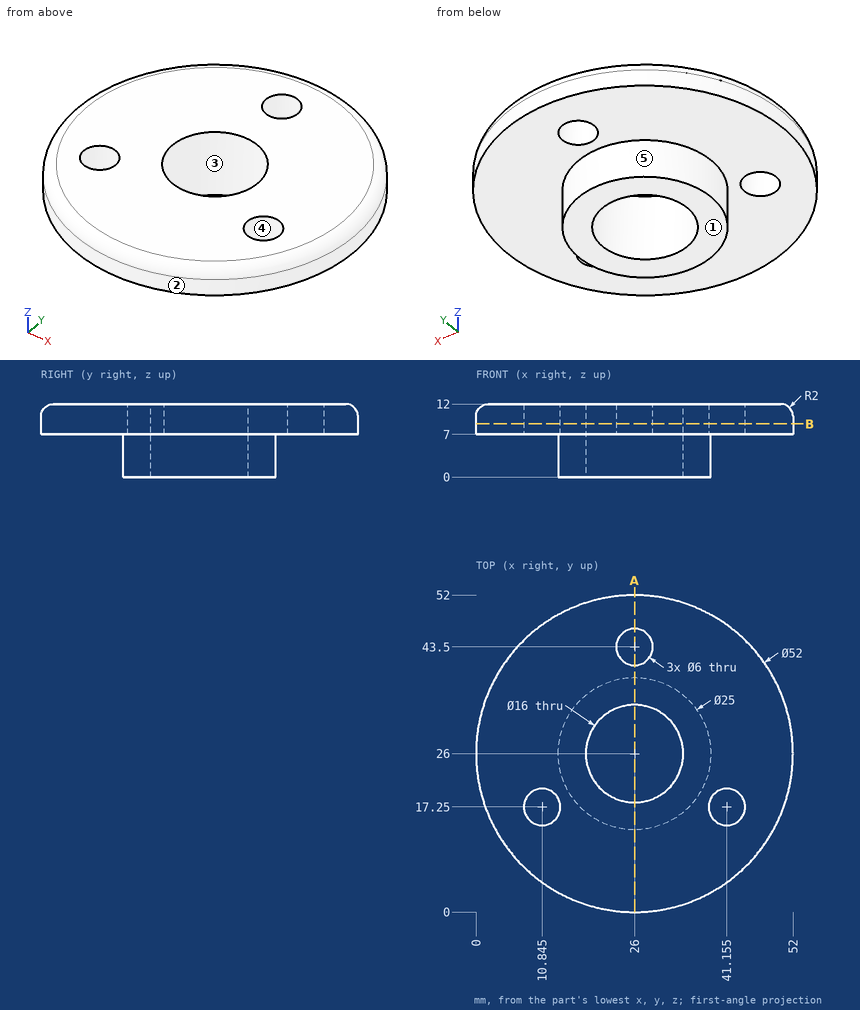
Here's the drawing with two shaded views (mm, measured from the low corner). I have some questions. A direction names the side the tool comes from. Coordinates: 2 decimals unless noted, no trailing zeros. Loops run counter-clockwise (first coordinate to the right, second up) from the corner with the lowest first, then second, coordinate; pieces in that order, holes last. Notation, with made-up numbers: (22.25, -38.5) -> (63.25, -38.5) arc R7 ccw to (63.25, -27.5) -> close; hole circle Ø8 at (36, 15.25). An arc over 180 degrees is marked (long way). Put each result on its own line as item: value. Start each with the question number.
Q1. For the marked faces 4 and 5, which set-ups out of +Z, -Z, +X, -X, +Y, -Y let a thin tool reach every point of the face, with its end or its side?
Q2. I want a section at B-B (z = 8.75). Count the separate pieces of the cut face and the enclosed holes in it, plus the area to 3 significant figures.
Q3. Thinking about a two-plate mould opening in X: for the marked faces 1, 2 and 3, which applies, pulls with the +X half, pulls with the -X half, needs draft (parallel to the pull), parting line crosses it, or undercut?
Q4. If I drill on line 1 (Y direction, x = 26, z = 8.2); line 2 (Y direction, x = 26, z = 10.6); line 3 (Y direction, x = 26, z = 3.5), over which ranges is the centre line in solid material (lowest first)? Write a range as [from, to].
Q5. I'm going to push flat-ended pins straight in: P1, Ø1.5, axis at x = 17.5, z = 3, coming from the +Y side; P2, Ø4, axis at x = 8.5, z = 10.5, coming from the +Y side (1 decimal). Where does each tip first touch, or does it pass through?
Q6. I want a section at A-A (x = 26). Write out the boundary of the cut face in (y, z), plus the area to 3 significant figures.
Taken from the geometry:
1. face 4: +Z, -Z
1. face 5: -Z
2. separate pieces: 1
2. enclosed holes: 4
2. area: 1,840 mm2
3. face 1: needs draft
3. face 2: parting line crosses it
3. face 3: undercut
4. line 1: y = [0, 18], [34, 40.5], [46.5, 52]
4. line 2: y = [0.09, 18], [34, 40.5], [46.5, 51.91]
4. line 3: y = [13.5, 18], [34, 38.5]
5. P1: stops at y = 35.81
5. P2: stops at y = 46.8
6. outline: (0, 7) -> (13.5, 7) -> (13.5, 0) -> (18, 0) -> (18, 12) -> (2, 12) arc R2 ccw to (0, 10) -> close; (34, 0) -> (38.5, 0) -> (38.5, 7) -> (40.5, 7) -> (40.5, 12) -> (34, 12) -> close; (46.5, 7) -> (52, 7) -> (52, 10) arc R2 ccw to (50, 12) -> (46.5, 12) -> close
6. area: 211 mm2
